Model file for the job. Use its own axes, mm. A direction names the side the tool comes from. Round coordinates to 2 decimals unless told otherwise and drop trailing zeros. Loops run counter-clockwise (first coordinate to the right, second up) from the corner with the lowest first, then second, coordinate; pieces in that order, holes last. Notation, with made-up numbers: (-1.75, 20.5) - (14.25, 20.5) arc R18 ccw to (14.25, 35.5) - close; hole circle Ø10 at (58, -3.75). An arc over 180 degrees is marked (long way). Answer as a JSON object with one key per item and string values.
from build123d import *

# Parameters (mm, degrees)
BOSS_EXTRUDE1_DEPTH = 20
CUT_EXTRUDE1_DEPTH  = 87.499082058
SKETCH5_R           = 1.75
SKETCH5_R_2         = 0.75
CUT_EXTRUDE2_DEPTH  = 87.499082058
FILLET1_R           = 2
SKETCH6_R           = 2.5
SKETCH6_R_2         = 1.25
SKETCH6_R_3         = 0.75
CUT_EXTRUDE3_DEPTH  = 20
SKETCH7_R           = 0.75
CUT_EXTRUDE4_DEPTH  = 20
SKETCH8_R           = 0.75
CUT_EXTRUDE5_DEPTH  = 20
FILLET2_R           = 2


with BuildPart() as part:
    # Sketch2 → Boss-Extrude1 (new body)
    with BuildSketch(Plane.XY):
        Polygon((4.868885541, 24.845866319), (4.868885541, 28.345866319), (65.368885541, 28.345866319), (65.368885541, -24.654133681), (4.868885541, -24.654133681), (4.868885541, -21.154133681), (61.868885541, -21.154133681), (61.868885541, 24.845866319), align=None)
    extrude(amount=-BOSS_EXTRUDE1_DEPTH)

    # Sketch3 → Cut-Extrude1 (cut, through all)
    with BuildSketch(Plane(origin=(0, 28.345866319, 0), x_dir=(1, 0, 0), z_dir=(0, 1, 0))):
        with BuildLine():
            ThreePointArc((14.868885541, 0), (7.79781773, 2.928932188), (4.868885541, 10))
            Line((4.868885541, 10), (4.868885541, 0))
            Line((4.868885541, 0), (14.868885541, 0))
        make_face()
        with BuildLine():
            ThreePointArc((4.868885541, 10), (7.79781773, 17.071067812), (14.868885541, 20))
            Line((14.868885541, 20), (4.868885541, 20))
            Line((4.868885541, 20), (4.868885541, 10))
        make_face()
    extrude(amount=-CUT_EXTRUDE1_DEPTH, mode=Mode.SUBTRACT)

    # Sketch5 → Cut-Extrude2 (cut, through all)
    with BuildSketch(Plane(origin=(0, 28.345866319, 0), x_dir=(1, 0, 0), z_dir=(0, 1, 0))):
        with Locations(Location((14.868885541, 10, 0), (0, 0, 270))):
            Circle(SKETCH5_R)
        with Locations(Location((20.868885541, 10, 0), (0, 0, 270))):
            Circle(SKETCH5_R)
        with Locations(Location((14.868885541, 4, 0), (0, 0, 270))):
            Circle(SKETCH5_R)
        with Locations(Location((8.868885541, 10, 0), (0, 0, 270))):
            Circle(SKETCH5_R)
        with Locations(Location((14.868885541, 16, 0), (0, 0, 270))):
            Circle(SKETCH5_R)
        with Locations(Location((19.111526229, 5.757359313, 0), (0, 0, 270))):
            Circle(SKETCH5_R_2)
        with Locations(Location((10.626244854, 5.757359313, 0), (0, 0, 270))):
            Circle(SKETCH5_R_2)
        with Locations(Location((10.626244854, 14.242640687, 0), (0, 0, 270))):
            Circle(SKETCH5_R_2)
        with Locations(Location((19.111526229, 14.242640687, 0), (0, 0, 270))):
            Circle(SKETCH5_R_2)
    extrude(amount=-CUT_EXTRUDE2_DEPTH, mode=Mode.SUBTRACT)

    # Fillet1
    fillet1_edges = [part.edges().sort_by_distance(p)[0] for p in [
        (65.368885541, 28.345866319, -10),
        (65.368885541, -24.654133681, -10),
    ]]
    fillet(fillet1_edges, radius=FILLET1_R)

    # Sketch6 → Cut-Extrude3 (cut)
    with BuildSketch(Plane(origin=(65.368885541, 0, 0), x_dir=(0, 0, -1), z_dir=(1, 0, 0))):
        with Locations((10, 1.845866319)):
            Circle(SKETCH6_R)
        with Locations((10, 7.845866319)):
            Circle(SKETCH6_R_2)
        with Locations((16, 1.845866319)):
            Circle(SKETCH6_R_2)
        with Locations((10, -4.154133681)):
            Circle(SKETCH6_R_2)
        with Locations((4, 1.845866319)):
            Circle(SKETCH6_R_2)
        with Locations((14.242640687, 6.088507006)):
            Circle(SKETCH6_R_3)
        with Locations((14.242640687, -2.396774369)):
            Circle(SKETCH6_R_3)
        with Locations((5.757359313, -2.396774369)):
            Circle(SKETCH6_R_3)
        with Locations((5.757359313, 6.088507006)):
            Circle(SKETCH6_R_3)
    extrude(amount=-CUT_EXTRUDE3_DEPTH, mode=Mode.SUBTRACT)

    # Sketch7 → Cut-Extrude4 (cut)
    with BuildSketch(Plane(origin=(65.368885541, 0, 0), x_dir=(0, 0, -1), z_dir=(1, 0, 0))):
        with Locations((16, 10.345866319)):
            Circle(SKETCH7_R)
        with Locations((4, 10.345866319)):
            Circle(SKETCH7_R)
        with Locations((4, -6.654133681)):
            Circle(SKETCH7_R)
        with Locations((16, -6.654133681)):
            Circle(SKETCH7_R)
    extrude(amount=-CUT_EXTRUDE4_DEPTH, mode=Mode.SUBTRACT)

    # Sketch8 → Cut-Extrude5 (cut)
    with BuildSketch(Plane(origin=(65.368885541, 0, 0), x_dir=(0, 0, -1), z_dir=(1, 0, 0))):
        with Locations((10, 17.845866319)):
            Circle(SKETCH8_R)
        with Locations((10, -14.154133681)):
            Circle(SKETCH8_R)
    extrude(amount=-CUT_EXTRUDE5_DEPTH, mode=Mode.SUBTRACT)

    # Fillet2
    fillet2_edges = [part.edges().sort_by_distance(p)[0] for p in [
        (61.868885541, -21.154133681, -10),
        (61.868885541, 24.845866319, -10),
    ]]
    fillet(fillet2_edges, radius=FILLET2_R)


solid = part.part
1) Probe probe 1 along X at (y, z) = (-22.7, -10); probe 2 along Y at (x, z) = (8.5, -8.25); probe 3 along Y at (x, z) = (62.65, -4). List the from-to ranges inside material, lowest first.
Values follow:
{"probe 1": "4.87 to 7.12, 10.62 to 13.12, 16.62 to 19.12, 22.62 to 65.37", "probe 2": "-24.65 to -21.15, 24.85 to 28.35", "probe 3": "-24.65 to -7.4, -5.9 to 0.6, 3.1 to 9.6, 11.1 to 28.35"}
2) Slice it at D-D on z = -1. List the corners of the cut face in (x, y).
Values follow:
{"outline": "(10.51, -24.65) - (63.37, -24.65) arc R2 ccw to (65.37, -22.65) - (65.37, 26.35) arc R2 ccw to (63.37, 28.35) - (10.51, 28.35) - (10.51, 24.85) - (59.87, 24.85) arc R2 cw to (61.87, 22.85) - (61.87, -19.15) arc R2 cw to (59.87, -21.15) - (10.51, -21.15) - close"}
3) Drop flat-ended pins along their axis: P1, Ø1.7, axis at x = 19.11, z = -5.76, coming from the -Y side; P2, Ø3, axis at y = 7.5, z = -8.5, coming from the -X side. Give the stop position or say it passes through.
Values follow:
{"P1": "y = -24.65", "P2": "x = 61.87"}
4) Slice it at B-B on z = -16. Count the separate pieces of the cut face and the enclosed holes in it, then the cut area to 3 significant figures.
Values follow:
{"separate pieces": "6", "enclosed holes": "0", "area": "527 mm²"}
5) Tool access for faces 5 (the flat face through (33, 24.846, -10)), 6 (the cylindrical face through (63.643, 5.423, -14.589)): list every direction of +Z, -Z, +X, -X, +Y, -Y with a clear straight run to the whole face (end or side of a thin tool).
Values follow:
{"face 5": "+Z, -Z, -X", "face 6": "+X, -X"}
6) Slice it at A-A on x = 24. List the corners of the cut face in (y, z).
Values follow:
{"outline": "(-24.65, -20) - (-21.15, -20) - (-21.15, 0) - (-24.65, 0) - close; (24.85, -20) - (28.35, -20) - (28.35, 0) - (24.85, 0) - close"}
7) Slice it at C-C on y = 12.5. List the corners of the cut face in (x, z), then the cut area to 3 significant figures.
Values follow:
{"outline": "(61.87, -20) - (65.37, -20) - (65.37, 0) - (61.87, 0) - close", "area": "70.0 mm²"}
8) Two-plate mould, pull along Z, no slides. Class faces 1 (the flat face through (63, 0, -20)), 2 (the cylindrical face through (18.446, 26.62, -5.411)), 3 (the cylindrical face through (11.259, 26.62, -5.354)), 4 (the flat face through (61.869, 1.6, -5.4)): pulls with the +Z half, pulls with the -Z half, needs draft (parallel to the pull), parting line crosses it, or undercut.
Values follow:
{"face 1": "pulls with the -Z half", "face 2": "undercut", "face 3": "undercut", "face 4": "needs draft"}
